Here's how the part is built. I have some questions about the finished solid (model axes, mm). A direction names the side the tool comes from. Give positions to 0.01 mm unless a question says otherwise; leave off trailing zeros. Loops run counter-clockwise (first coordinate to the right, second up) from the corner with the lowest first, then second, coordinate; pieces in that order, holes last. Notation, with made-up numbers: (-22, 42) -> (-7, 42) arc R12 cw to (-7, 55) -> close; hole circle Ø7 at (24, -14). An arc over 180 degrees is marked (long way). Answer in a Markdown table with one row per item. Add a question column.
Item 1: If I drill on line 1 (Z direction, x = 0, y = -22); line 2 (X direction, y = -0.5, z = 76); line 3 (Y direction, x = 0, z = -13), over which ranges is the centre line in solid material (lowest first)?
Item 2: Which directions (+Z, -Z, +X, -X, +Y, -Y) give clear straight access to the entire face, cutting with the end or side of a thin tool? Please do faces 1 (the face through (-28.995, 0.531, 93.67)), 2 (the face through (0, -23, 50)), 3 (the face through (28.995, -0.531, 93.67)).
Item 3: If we section it at D-D (y = 0): Write out the boundary of the cut face in (x, z), then the cut area to 3 significant figures.
Item 4: For P1, Ø12, axis at x = -11.5, z = 39.5, coming from the -Y side; P2, Ø10, axis at x = 23.5, z = 72.5, coming from the -Y side; P3, Ø8, axis at x = -10.5, y = 18, coming from the -Z side, each with a flat end and sliding along its axis, tell me the tip position at first contact or that it passes through.
Item 5: We'd pull the mould along Y, two halves only. Please class faces 4 (the face through (23.977, 1.055, -13.647)), 5 (the face through (0, -28, 96)), 6 (the face through (0, 0, 180)), 7 (the face through (-2.87, -22.1, 136.93)): released by +Y, released by -Y, zero draft, split by the parting line, or undercut.
Item 6: If we section it at C-C (z = 172.5): Write out the boundary of the cut face in (x, y).
Item 7: If we section it at B-B (z = 130): Write out the boundary of the cut face in (x, y).
Item 8: If we section it at A-A (x = 0): Give the number of separate pieces and of enclosed holes in the cut face, then the cut area to 3 significant figures.
```python
from build123d import *

# Parameters (mm, degrees)
SKETCH1_R           = 29
BOSS_EXTRUDE1_DEPTH = 190
SKETCH2_R           = 30
BOSS_EXTRUDE2_DEPTH = 25
SKETCH4_OUTSIDE_W   = 108.228
SKETCH4_OUTSIDE_H   = 108.228
SKETCH4_OUTSIDE_W_2 = 84.198703348
SKETCH4_OUTSIDE_H_2 = 56
CUT_EXTRUDE1_DEPTH  = 190
SKETCH5_R           = 24
CUT_EXTRUDE2_DEPTH  = 22
SKETCH6_R           = 24.1
CUT_EXTRUDE3_DEPTH  = 3
SKETCH7_R           = 18
CUT_EXTRUDE4_DEPTH  = 180
SKETCH8_R           = 5
SKETCH8_R_2         = 7.5
CUT_EXTRUDE5_DEPTH  = 180
CHAMFER1_SIZE       = 1


with BuildPart() as part:
    # Sketch1 → Boss-Extrude1 (new body)
    with BuildSketch(Plane.XY):
        Circle(SKETCH1_R)
    extrude(amount=BOSS_EXTRUDE1_DEPTH)

    # Sketch2 → Boss-Extrude2 (add)
    with BuildSketch(Plane(origin=(0, 0, 0), x_dir=(-1, 0, 0), z_dir=(0, 0, -1))):
        Circle(SKETCH2_R)
    extrude(amount=BOSS_EXTRUDE2_DEPTH)

    # Sketch4 outside → Cut-Extrude1 (cut)
    with BuildSketch(Plane.XY.offset(190)):
        Rectangle(SKETCH4_OUTSIDE_W, SKETCH4_OUTSIDE_H)
        Rectangle(SKETCH4_OUTSIDE_W_2, SKETCH4_OUTSIDE_H_2, mode=Mode.SUBTRACT)
    extrude(amount=-CUT_EXTRUDE1_DEPTH, mode=Mode.SUBTRACT)

    # Sketch5 → Cut-Extrude2 (cut)
    with BuildSketch(Plane(origin=(0, 0, -25), x_dir=(-1, 0, 0), z_dir=(0, 0, -1))):
        Circle(SKETCH5_R)
    extrude(amount=-CUT_EXTRUDE2_DEPTH, mode=Mode.SUBTRACT)

    # Sketch6 → Cut-Extrude3 (cut)
    with BuildSketch(Plane(origin=(0, 0, -3), x_dir=(-1, 0, 0), z_dir=(0, 0, -1))):
        Circle(SKETCH6_R)
    extrude(amount=-CUT_EXTRUDE3_DEPTH, mode=Mode.SUBTRACT)

    # Sketch7 → Cut-Extrude4 (cut)
    with BuildSketch(Plane(origin=(0, 0, 0), x_dir=(-1, 0, 0), z_dir=(0, 0, -1))):
        Circle(SKETCH7_R)
    extrude(amount=-CUT_EXTRUDE4_DEPTH, mode=Mode.SUBTRACT)

    # Sketch8 → Cut-Extrude5 (cut)
    with BuildSketch(Plane(origin=(0, 0, 0), x_dir=(1, 0, 0), z_dir=(0, 1, 0))):
        with Locations(Location((0, -55, 0), (0, 0, 270))):
            Circle(SKETCH8_R)
        with Locations(Location((0, -130, 0), (0, 0, 270))):
            Circle(SKETCH8_R_2)
    extrude(amount=-CUT_EXTRUDE5_DEPTH, mode=Mode.SUBTRACT)

    # Chamfer1
    chamfer1_edges = [part.edges().sort_by_distance(p)[0] for p in [
        (24, 0, -25),
    ]]
    chamfer(chamfer1_edges, length=CHAMFER1_SIZE)


solid = part.part
```
Recorded:
| question | item | result |
|---|---|---|
| 1 | line 1 | z = 0 to 50, 60 to 122.5, 137.5 to 190 |
| 1 | line 2 | x = -29 to -17.99, 17.99 to 29 |
| 1 | line 3 | y = -30 to -24, 24 to 30 |
| 2 | face 1 | +Z, -X |
| 2 | face 2 | -Y |
| 2 | face 3 | +Z, +X |
| 3 | outline | (-30, -25) -> (-25, -25) -> (-24, -24) -> (-24, -3) -> (-24.1, -3) -> (-24.1, 0) -> (-18, 0) -> (-18, 180) -> (18, 180) -> (18, 0) -> (24.1, 0) -> (24.1, -3) -> (24, -3) -> (24, -24) -> (25, -25) -> (30, -25) -> (30, 0) -> (29, 0) -> (29, 190) -> (-29, 190) -> (-29, 0) -> (-30, 0) -> close |
| 3 | area | 4,840 mm^2 |
| 4 | P1 | stops at y = -28 |
| 4 | P2 | stops at y = -22.33 |
| 4 | P3 | stops at z = -24.84 |
| 5 | face 4 | undercut |
| 5 | face 5 | released by -Y |
| 5 | face 6 | undercut |
| 5 | face 7 | zero draft |
| 6 | outline | (-7.55, -28) -> (7.55, -28) arc R29 ccw to (7.55, 28) -> (-7.55, 28) arc R29 ccw to start; hole circle Ø36 at (0, 0) |
| 7 | outline | (-7.55, -28) -> (-7.5, -28) -> (-7.5, -16.36) arc R18 cw (long way) to (7.5, -16.36) -> (7.5, -28) -> (7.55, -28) arc R29 ccw to (7.55, 28) -> (-7.55, 28) arc R29 ccw to start |
| 8 | separate pieces | 3 |
| 8 | enclosed holes | 0 |
| 8 | area | 4,210 mm^2 |
